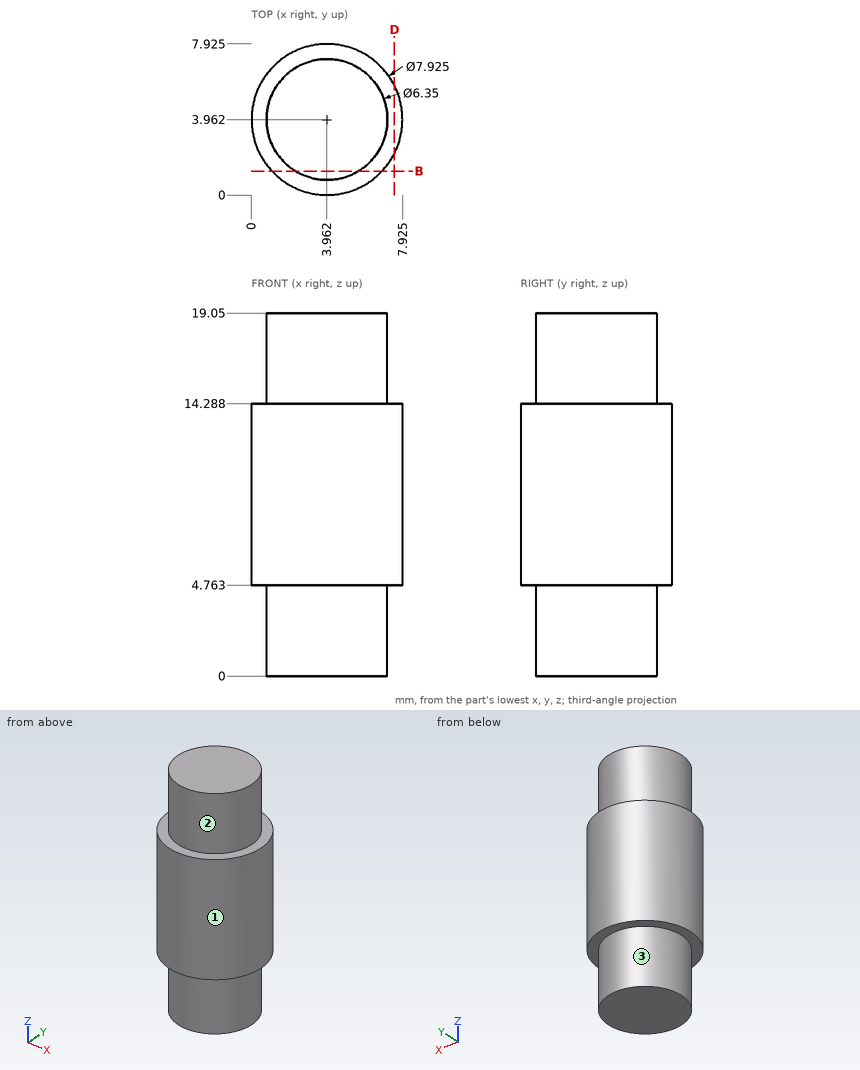
Verification items for this drawing (mm, ordinates from the low corner). A direction names the side the tool comes from. Coordinates: 2 decimals unless noted, no trailing zeros. Loops run counter-clockwise (first coordinate to the right, second up) from the corner with the lowest first, then second, coordinate; pieces in that order, holes last. Notation, with made-up numbers: (32, 71) - (50, 71) arc R29 cw to (50, 108) - close; hole circle Ø6 at (23, -20). An arc over 180 degrees is marked (long way). Use one line per item in the form item = value. Start each with the question number.
Item 1: Gauge pin test, flat ends, axial feed: pin 1 (2 mm diameter, centred on x = 5, z = 2.5, fed in from -Y); pin 2 (2 mm diameter, centred on y = 6, z = 14.5, fed in from -X) (1 decimal); pin 3 (1 mm diameter, centred on y = 3.5, z = 11.5, fed in from +X) (1 decimal); pin 4 (1 mm diameter, centred on y = 4, z = 15.5, fed in from -X). Record the tip position at first contact, or that the pin passes through.
Item 2: Section check B-B, the plane y = 1.25. Enter the section's corners in (x, z).
Item 3: Tool access check on the marked faces 1, 2 and 3. Record the directions out of +Z, -Z, +X, -X, +Y, -Y that give a thin tool (end or side, any length) a straight path to the whole face; none if there is none.
Item 4: Section check D-D, the plane x = 7.5. Enter the section's corners in (y, z), and give its area (3 significant figures).
Item 5: Thickness scan on probe 1 along Z at (x, y) = (4.75, 0.75); probe 2 along Y at (x, z) = (2.25, 3.75) (1 decimal); probe 3 along Y at (x, z) = (2, 5.25) (1 decimal). Record the ranges inside material, lowest first.
Computed:
q1.pin_1 = 0.79
q1.pin_2 = 0.1
q1.pin_3 = 7.9
q1.pin_4 = 0.79
q2.outline = (1.07, 4.76) - (2.31, 4.76) - (2.31, 0) - (5.61, 0) - (5.61, 4.76) - (6.85, 4.76) - (6.85, 14.29) - (5.61, 14.29) - (5.61, 19.05) - (2.31, 19.05) - (2.31, 14.29) - (1.07, 14.29) - close
q3.face_1 = +Z, -Z
q3.face_2 = +Z
q3.face_3 = -Z
q4.outline = (2.18, 4.76) - (5.75, 4.76) - (5.75, 14.29) - (2.18, 14.29) - close
q4.area = 34.0 mm2
q5.probe_1 = 4.76 to 14.29
q5.probe_2 = 1.3 to 6.6
q5.probe_3 = 0.5 to 7.4
